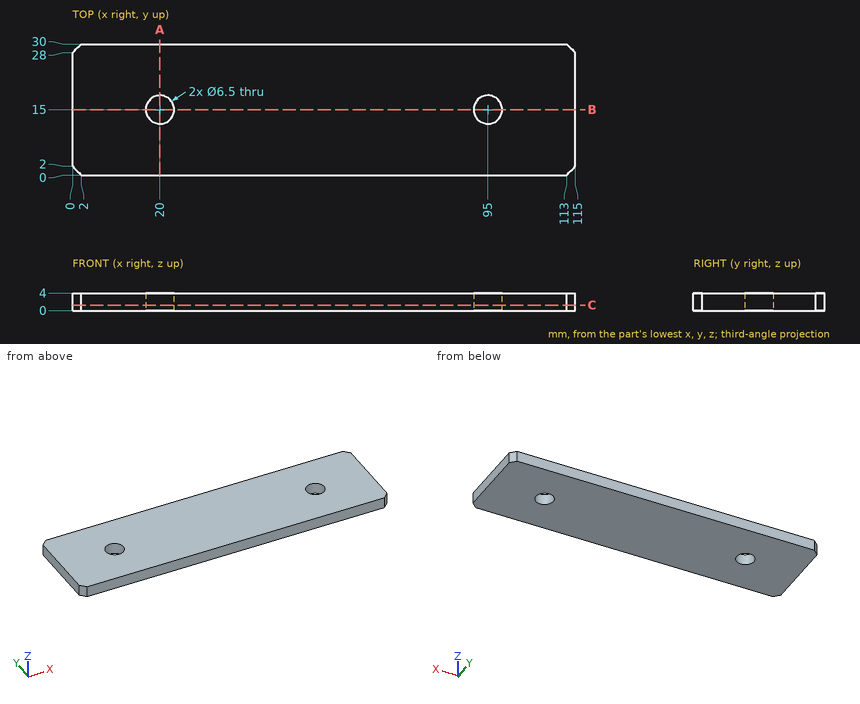
The drawing under review shows one solid part. Ordinate dimensions are in mm from its lowest x, y, z. Coordinates: 2 decimals unless noted, no trailing zeros. Order: outer loops, then holes, each group sorted by start corner. A loop starts at its lowest first (then second) coordinate and runs counter-clockwise, first axis right, second up. Notation, with made-up numbers: (21.25, 60) -> (67.25, 60) arc R25 cw to (67.25, 93) -> close; hole circle Ø8 at (-4, -28). An arc over 180 degrees is marked (long way). Answer as CSV lines item,"result".
Q1. Clearance check with a flat-ended pin moving along its axis: pin 1 Ø6 at (x, y) = (95, 15) entering from +Z. State where the tip first meets the part, or that it passes through.
Model answer:
pin 1,"passes through"
Q2. We need section C-C (z = 1.25). State the section outline as (x, y) points, plus the area to 3 significant figures.
Model answer:
outline,"(0, 2) -> (2, 0) -> (113, 0) -> (115, 2) -> (115, 28) -> (113, 30) -> (2, 30) -> (0, 28) -> close; hole circle Ø6.5 at (20, 15); hole circle Ø6.5 at (95, 15)"
area,"3,380 mm2"
Q3. We need section B-B (y = 15). State the section outline as (x, z) points.
Model answer:
outline,"(0, 0) -> (16.75, 0) -> (16.75, 4) -> (0, 4) -> close; (23.25, 0) -> (91.75, 0) -> (91.75, 4) -> (23.25, 4) -> close; (98.25, 0) -> (115, 0) -> (115, 4) -> (98.25, 4) -> close"
Q4. Wall thickness on line 1 along Y through (x, z) = (20, 2.05); line 2 along X through (y, z) = (16.75, 2.25); line 3 along Y through (x, z) = (21, 3.8): over which ranges is each line inside the solid? List them lowest first. Write a range as [from, to].
Model answer:
line 1,"y = [0, 11.75], [18.25, 30]"
line 2,"x = [0, 17.26], [22.74, 92.26], [97.74, 115]"
line 3,"y = [0, 11.91], [18.09, 30]"
Q5. We need section A-A (x = 20). State the section outline as (y, z) points, plus the area to 3 significant figures.
Model answer:
outline,"(0, 0) -> (11.75, 0) -> (11.75, 4) -> (0, 4) -> close; (18.25, 0) -> (30, 0) -> (30, 4) -> (18.25, 4) -> close"
area,"94.0 mm2"
